from build123d import *

# Parameters (mm, degrees)
BOSS_EXTRUDE1_START      = -260
BOSS_EXTRUDE1_DEPTH      = 260
BOSS_EXTRUDE4_DEPTH      = 24
BOSS_EXTRUDE5_REACH      = 2447.334
BOSS_EXTRUDE5_END_RADIUS = 20
SKETCH5_R                = 5
FILLET1_R                = 2
FILLET2_R                = 2
CHAMFER2_SIZE            = 1


with BuildPart() as part:
    # Sketch1 → Boss-Extrude1 (new body)
    with BuildSketch(Plane(origin=(83.573308801, 222.892709782, 0), x_dir=(0.9363450005078556, -0.3510812441927706, 0), z_dir=(-0.3510812441927706, -0.9363450005078556, 0)).offset(BOSS_EXTRUDE1_START)):
        with BuildLine():
            ThreePointArc((546.192823225, 2320.014515708), (561.248526003, 2335.070218486), (546.192823225, 2350.125921264))
            ThreePointArc((546.192823225, 2350.125921264), (531.137120447, 2335.070218486), (546.192823225, 2320.014515708))
        make_face()
    extrude(amount=BOSS_EXTRUDE1_DEPTH)



with BuildPart() as body_2:
    # Sketch6 → Boss-Extrude4 (new body)
    with BuildSketch(Plane(origin=(0, 0, 2323.070218486), x_dir=(-1, 0, 0), z_dir=(0, 0, -1))):
        with BuildLine():
            ThreePointArc((-589.676062924, -40.026603584), (-563.92753803, -51.73187871), (-552.222262904, -25.983353816))
            ThreePointArc((-552.222262904, -25.983353816), (-577.970787798, -14.27807869), (-589.676062924, -40.026603584))
        make_face()
        with BuildLine():
            ThreePointArc((-582.18530292, -37.21795363), (-566.736188003, -44.241118713), (-559.713022893, -28.792003808))
            ThreePointArc((-559.713022893, -28.792003808), (-575.162137825, -21.768838687), (-582.18530292, -37.21795363))
        make_face(mode=Mode.SUBTRACT)
    extrude(amount=-BOSS_EXTRUDE4_DEPTH)


with BuildPart() as part_1:
    add(part.part)

    add(body_2.part)  # Boss-Extrude5 merges body 2
    # Boss-Extrude5: up to this cylinder (the profile starts outside it)
    boss_extrude5_end = Plane(origin=(570.949162914, -33.0049787, 2335.070218), z_dir=(0, 0, -1)) * Cylinder(BOSS_EXTRUDE5_END_RADIUS, 4935.668, mode=Mode.PRIVATE)
    # Sketch5 → Boss-Extrude5 (add, up to the surface)
    with BuildSketch(Plane(origin=(83.573308801, 222.892709782, 0), x_dir=(0.9363450005078556, -0.3510812441927706, 0), z_dir=(-0.3510812441927706, -0.9363450005078556, 0)), mode=Mode.PRIVATE) as boss_extrude5_sk1:
        with Locations(Location((546.192823225, 2335.070218486, 0), (0, 0, 180))):
            Circle(SKETCH5_R)
    boss_extrude5_tool1 = extrude(boss_extrude5_sk1.sketch, amount=BOSS_EXTRUDE5_REACH, mode=Mode.PRIVATE) - boss_extrude5_end
    add(boss_extrude5_tool1.solids().sort_by_distance((594.998228, 31.134654, 2335.070218))[0])

    # Fillet1
    fillet1_edges = [part_1.edges().sort_by_distance(p)[0] for p in [
        (582.429546976, -16.628141955, 2335.070218486),
    ]]
    fillet(fillet1_edges, radius=FILLET1_R)

    # Fillet2
    fillet2_edges = [part_1.edges().sort_by_distance(p)[0] for p in [
        (559.713022908, -28.79200377, 2347.070218486),
        (589.676062924, -40.026603584, 2347.070218486),
        (559.713022908, -28.79200377, 2323.070218486),
        (589.676062924, -40.026603584, 2323.070218486),
    ]]
    fillet(fillet2_edges, radius=FILLET2_R)

    # Chamfer2
    chamfer2_edges = [part_1.edges().sort_by_distance(p)[0] for p in [
        (599.679953144, 29.379247614, 2335.070218486),
    ]]
    chamfer(chamfer2_edges, length=CHAMFER2_SIZE)


solid = part_1.part
The model under review builds one solid part; all positions refer to its coordinate system, in mm. Round coordinates to 2 decimals unless told otherwise and drop trailing zeros. Answer as CSV lines item,"result". Start each with the question number.
Q1. Clearance check with flat-ended pins moving along their axes: P1, Ø1.5, axis at y = 230, z = 2346.5, coming from the +X side; P2, Ø1, axis at y = 142.5, z = 2328, coming from the -X side; P3, Ø12, axis at y = 210, z = 2344.5, coming from the -X side. State where each tip first meets the part, or that it passes through.
Q2. Wall thickness on line 1 along Z through (x, y) = (663, 205.5); line 2 along X through (y, z) = (211, 2325); line 3 along X through (y, z) = (150, 2337.5): over which ranges is each line inside the solid? List them lowest first.
Q3. The part is to be moulded in two halves that separate along X. For faces 1 (the face through (686.08, 274.66, 2335.28)), 2 (the face through (594.8, 31.21, 2328.59)), 3 (the face through (562, -44, 2347.07)), say which applies: +X half, -X half, draft (parallel to the pull), parting line (faces both ways), or undercut.
Result set:
1,P1,"stops at x = 680.94"
1,P2,"stops at x = 622.23"
1,P3,"stops at x = 645.38"
2,line 1,"z = 2320.22 to 2349.92"
2,line 2,"x = 650.49 to 674.39"
2,line 3,"x = 623.7 to 655.44"
3,face 1,"+X half"
3,face 2,"undercut"
3,face 3,"draft"
